CAD build for the part. Positions are in the model's coordinates, mm. A direction names the side the tool comes from. Give positions to 0.01 mm unless a question says otherwise; leave off trailing zeros. Order: outer loops, then holes, each group sorted by start corner. A loop starts at its lowest first (then second) coordinate and runs counter-clockwise, first axis right, second up. Notation, with made-up numbers: M -19,-35.75 L -8,-35.75 A21 ccw -8,-31.75 Z; hole C 27.25,-6.75 d6. An arc over 180 degrees is marked long. Put each result on its own line as item: value. Start each with the question number.
1) Cut at C-C (y = 1). Write the cut outline in (x, z) (3 decimals).
2) Cut at B-B (x = 80). Write the cut outline in (y, z) (3 decimals), and give its area (3 significant figures).
3) Tool access for faces 5 (the face through (0, -7, -49)), 6 (the face through (49, 4, -4.775)): list every direction of +Z, -Z, +X, -X, +Y, -Y with a clear straight run to the whole face (end or side of a thin tool).
4) Drill centre lines: line 1 (Z direction, x = 33.5, y = 94.5) (3 decimals); line 2 (X direction, y = 271, z = -58); line 3 (X direction, y = -27.5, z = -87.5). Where is each one in solid material? Low to high. Write a range as [from, to].
5) Cut at A-A (z = -43). Write the cut outline in (x, y), and give its area (3 significant figures).
6) Two-plate mould, pull along Z, no slides. Class faces 1 (the face through (51, 4, -92.175)), 2 (the face through (6.3, -6, -49)), 3 (the face through (49, 4, 1.525)), 4 (the face through (94, -361.5, -49)): released by +Z, released by -Z, zero draft, split by the parting line, or undercut.
```python
from build123d import *

# Parameters (mm, degrees)
BOSS_EXTRUDE1_DEPTH = 361.5
CUT_EXTRUDE1_REACH  = 390.178


with BuildPart() as part:
    # Sketch2 → Boss-Extrude1 (new, symmetric)
    with BuildSketch(Plane(origin=(0, 0, 0), x_dir=(1, 0, 0), z_dir=(0, 1, 0))):
        with BuildLine():
            Line((7.875, -1.525), (92.125, -1.525))
            ThreePointArc((92.125, -1.525), (97.693465902, 0.781534098), (100, 6.35))
            Line((100, 6.35), (100, 90.6))
            ThreePointArc((100, 90.6), (97.693465902, 96.168465902), (92.125, 98.475))
            Line((92.125, 98.475), (7.875, 98.475))
            ThreePointArc((7.875, 98.475), (2.306534098, 96.168465902), (0, 90.6))
            Line((0, 90.6), (0, 6.35))
            ThreePointArc((0, 6.35), (2.306534098, 0.781534098), (7.875, -1.525))
        make_face()
        with BuildLine():
            Line((12.6, 4.775), (87.4, 4.775))
            ThreePointArc((87.4, 4.775), (91.854772721, 6.620227279), (93.7, 11.075))
            Line((93.7, 11.075), (93.7, 85.875))
            ThreePointArc((93.7, 85.875), (91.854772721, 90.329772721), (87.4, 92.175))
            Line((87.4, 92.175), (12.6, 92.175))
            ThreePointArc((12.6, 92.175), (8.145227279, 90.329772721), (6.3, 85.875))
            Line((6.3, 85.875), (6.3, 11.075))
            ThreePointArc((6.3, 11.075), (8.145227279, 6.620227279), (12.6, 4.775))
        make_face(mode=Mode.SUBTRACT)
    extrude(amount=BOSS_EXTRUDE1_DEPTH, both=True)

    # Sketch4 → Cut-Extrude1 (cut, up to next)
    with BuildSketch(Plane.XY.offset(1.525), mode=Mode.PRIVATE) as cut_extrude1_sk1:
        Polygon((100, 361.5), (0, 338.5), (0, 361.5), align=None)
    cut_extrude1_tool1 = extrude(cut_extrude1_sk1.sketch, amount=-CUT_EXTRUDE1_REACH, mode=Mode.PRIVATE) & part.part
    add(cut_extrude1_tool1.solids().sort_by_distance((33.333333, 353.833333, 1.525))[0], mode=Mode.SUBTRACT)


solid = part.part
```
Solution:
1. outline: M 0,-90.6 A7.875 ccw 7.875,-98.475 L 92.125,-98.475 A7.875 ccw 100,-90.6 L 100,-6.35 A7.875 ccw 92.125,1.525 L 7.875,1.525 A7.875 ccw 0,-6.35 Z; hole M 6.3,-85.875 A6.3 ccw 12.6,-92.175 L 87.4,-92.175 A6.3 ccw 93.7,-85.875 L 93.7,-11.075 A6.3 ccw 87.4,-4.775 L 12.6,-4.775 A6.3 ccw 6.3,-11.075 Z
2. outline: M -361.5,-98.475 L 356.9,-98.475 L 356.9,-92.175 L -361.5,-92.175 Z; M -361.5,-4.775 L 356.9,-4.775 L 356.9,1.525 L -361.5,1.525 Z
2. area: 9,050 mm²
3. face 5: +Z, -Z, -X, +Y, -Y
3. face 6: +Y, -Y
4. line 1: [-98.475, -92.175], [-4.775, 1.525]
4. line 2: [0, 6.3], [93.7, 100]
4. line 3: [0, 6.51], [93.49, 100]
5. outline: M 0,-361.5 L 6.3,-361.5 L 6.3,339.95 L 0,338.5 Z; M 93.7,-361.5 L 100,-361.5 L 100,361.5 L 93.7,360.05 Z
5. area: 8,960 mm²
6. face 1: undercut
6. face 2: undercut
6. face 3: released by +Z
6. face 4: zero draft
